```python
from build123d import *

# Parameters (mm, degrees)
SKETCH_1_W                = 12
SKETCH_1_H                = 8
EXTRUDE_1_DEPTH           = 350
CHAMFER_1_SIZE            = 0.5
CHAMFER_2_SIZE            = 0.5
HOLE_WIZARD_1_D           = 3.4
HOLE_WIZARD_1_CBORE_D     = 6
HOLE_WIZARD_1_CBORE_DEPTH = 3.4
PATTERN_LINEAR_1_COUNT    = 14
PATTERN_LINEAR_1_PITCH    = 25


with BuildPart() as part:
    # 草图1 → 凸台-拉伸1 (new body)
    with BuildSketch(Plane.XY):
        Rectangle(SKETCH_1_W, SKETCH_1_H)
    extrude(amount=EXTRUDE_1_DEPTH)

    # 倒角1
    chamfer_1_edges = [part.edges().sort_by_distance(p)[0] for p in [
        (6, 4, 175),
    ]]
    chamfer(chamfer_1_edges, length=CHAMFER_1_SIZE)

    # 倒角2
    chamfer_2_edges = [part.edges().sort_by_distance(p)[0] for p in [
        (-6, 4, 175),
    ]]
    chamfer(chamfer_2_edges, length=CHAMFER_2_SIZE)

    # 打孔尺寸根据内六角圆柱头螺钉的类型1 (through all)
    with Locations(Plane(origin=(0, 4, 0), x_dir=(1, 0, 0), z_dir=(0, 1, 0))):
        with Locations((0, -12.5)):
            hole_wizard_1 = CounterBoreHole(HOLE_WIZARD_1_D / 2, HOLE_WIZARD_1_CBORE_D / 2, HOLE_WIZARD_1_CBORE_DEPTH)

    # 阵列(线性)1: 打孔尺寸根据内六角圆柱头螺钉的类型1 ×14
    with Locations(*[(0, 0, i * PATTERN_LINEAR_1_PITCH) for i in range(1, PATTERN_LINEAR_1_COUNT)]):
        add(hole_wizard_1, mode=Mode.SUBTRACT)


solid = part.part
```
The model under review builds one solid part; all positions refer to its coordinate system, in mm. A direction names the side the tool comes from. Give positions to 0.01 mm unless a question says otherwise; leave off trailing zeros. Write each question's results on one line, items separated by ' | '. Start each with the question number.
1. For probe 1 along X at (y, z) = (2.3, 62.5); probe 2 along Y at (x, z) = (2, 162); probe 3 along X at (y, z) = (3.75, 286.5), list the stretches that pass through material, from the lowest coordinate up. Write a range as [from, to].
2. For faces 5 (the cylindrical face through (-0.391, 2.324, 184.526)), 6 (the flat face through (0, -4, 173)), list the 3-axis set-ups (+Z, -Z, +X, -X, +Y, -Y) from which the entire face can be reached by the end or side of a thin tool; tool diameter is ignored.
3. We need section A-A (y = -2.5). Count the separate pieces of the cut face and the enclosed holes in it, and give its area (3 significant figures).
4. Insertion check: pin 1 Ø4 at (x, z) = (0, 287.5) entering from +Y; pin 2 Ø4 at (x, y) = (3.5, -0.5) entering from -Z. Each pin has a flat end and moves straight along its axis. Give the tip position at first contact, or say it passes through.
5. Mouldability with a two-part tool opening along X and no side actions: class faces 1 (the flat face through (2, 0.6, 62)), 2 (the flat face through (6, 0, 173)), 3 (the cylindrical face through (-0.65, 2.32, 15.43)), 4 (the flat face through (0, 4, 173)) as released by +X, released by -X, zero draft, split by the parting line, or undercut.
Results found:
1) probe 1: x = [-6, -3], [3, 6] | probe 2: y = [-4, 0.6] | probe 3: x = [-5.75, -2.83], [2.83, 5.75]
2) face 5: +Y | face 6: +Z, -Z, +X, -X, -Y
3) separate pieces: 1 | enclosed holes: 14 | area: 4,070 mm^2
4) pin 1: stops at y = 0.6 | pin 2: stops at z = 0
5) face 1: undercut | face 2: released by +X | face 3: undercut | face 4: zero draft
